from build123d import *

# Parameters (mm, degrees)
FILLET1_R = 10


with BuildPart() as part:
    # Sketch1 → Revolve1 (revolve)
    with BuildSketch(Plane(origin=(0, 0, 0), x_dir=(1, 0, 0), z_dir=(0, 1, 0)), mode=Mode.PRIVATE) as revolve1_sk:
        Polygon((0, 200), (0, 227.5), (14, 227.5), (14, 220), (41, 220), (41, 203), (27, 203), (27, 189), (41, 189), (41, 177), (27, 177), (27, 163), (41, 163), (41, 151), (14, 151), (14, 200), align=None)
    revolve(revolve1_sk.sketch.rotate(Axis((0, 0, 0), (1, 0, 0)), 180), axis=Axis((0, 0, 0), (1, 0, 0)))

    # Fillet1
    fillet1_edges = [part.edges().sort_by_distance(p)[0] for p in [
        (14, 0, -200),
    ]]
    fillet(fillet1_edges, radius=FILLET1_R)


solid = part.part
Here's how the part is built. I have some questions about the finished solid (model axes, mm). A direction names the side the tool comes from. Give positions to 0.01 mm unless a question says otherwise; leave off trailing zeros. Order: outer loops, then holes, each group sorted by start corner. A loop starts at its lowest first (then second) coordinate and runs counter-clockwise, first axis right, second up. Notation, with made-up numbers: M 74,-32.5 L 84,-32.5 A35 ccw 84,-0.5 Z; hole C 88,-24 d8. An arc over 180 degrees is marked long. Answer as a JSON object with one key per item and string values. Group by question number.
1) Please list where these lines run through material, in increasing order: L1, parallel to Y at x = 37.25, z = 0; L2, parallel to Z at x = 27.5, y = -15; L3, parallel to Z at x = 30, y = 53.5. Write a range as [from, to].
2) On a 3-axis mill with a long thin cutter (end or side, diameter ignored), from which of +Z, -Z, +X, -X, +Y, -Y can I reach the whole of each face in a straight line? I mean faces 1 (the flat face through (14, -142, -55)), 2 (the flat face through (41, 195, 64)), 3 (the cylindrical face through (27.689, 195.178, 101.517)). Say none if no direction works.
3) We'd pull the mould along Z, two halves only. Please class faces 4 (the cylindrical face through (7.098, -68.335, 216.994)), 5 (the flat face through (0, 201, 1)), 6 (the cylindrical face through (27.311, -45.356, 144.027)): pulls with the +Z half, pulls with the -Z half, needs draft (parallel to the pull), parting line crosses it, or undercut.
4) I'm going to push flat-ended pins straight in: pin 1 Ø1.5 at (x, y) = (13.5, -7.5) entering from -Z; pin 2 Ø4 at (x, y) = (12, -179.5) entering from +Z; pin 3 Ø10 at (x, y) = (6, -126.5) entering from +Z; pin 4 Ø10 at (y, z) = (-150, 170.5) entering from -X. Where does each tip first touch, or does it pass through?
5) Suppose I cut it at A-A, the plane x = 34. Write out the boundary of the cut face in (y, z), plus the area to 3 significant figures.
Results found:
{
 "1": {"L1": "[-220, -203], [-189, -177], [-163, -151], [151, 163], [177, 189], [203, 220]", "L2": "[-219.49, -202.45], [-188.4, -176.36], [-162.31, -150.25], [150.25, 162.31], [176.36, 188.4], [202.45, 219.49]", "L3": "[-213.4, -195.82], [-181.27, -168.72], [-153.97, -141.2], [141.2, 153.97], [168.72, 181.27], [195.82, 213.4]"},
 "2": {"face 1": "-X", "face 2": "+Z, -Z, +X, +Y, -Y", "face 3": "+X"},
 "3": {"face 4": "parting line crosses it", "face 5": "needs draft", "face 6": "undercut"},
 "4": {"pin 1": "z = -227.4", "pin 2": "z = 142.3", "pin 3": "z = 192.34", "pin 4": "x = 0"},
 "5": {"outline": "C 0,0 d440; C 0,0 d378; C 0,0 d326; hole C 0,0 d406; hole C 0,0 d354; hole C 0,0 d302", "area": "48,200 mm²"}
}
